```python
from build123d import *


with BuildPart() as part:
    # Sketch1 → Revolve1 (revolve)
    with BuildSketch(Plane.XY):
        Polygon((0, 0), (0, 3.5), (3.91, 3.5), (3.91, 1.4), (32.91, 1.4), (32.91, 1.9), (38.91, 1.9), (38.91, 0), align=None)
    revolve(axis=Axis((38.91, 0, 0), (-1, 0, 0)))


solid = part.part
```
Geometry check sheet. Reference: the model listing, model coordinates, mm. A direction names the side the tool comes from. Round coordinates to 2 decimals unless told otherwise and drop trailing zeros. Order: outer loops, then holes, each group sorted by start corner. A loop starts at its lowest first (then second) coordinate and runs counter-clockwise, first axis right, second up. Notation, with made-up numbers: M 19,-5.75 L 77,-5.75 A5 cw 77,2.25 Z; hole C 86.25,-9 d5. An arc over 180 degrees is marked long. Write item = value, one per line.
Q1. Section check D-D (z = 3). Enter the section's corners in (x, y).
Answer block:
outline = M 0,-1.8 L 3.91,-1.8 L 3.91,1.8 L 0,1.8 Z
Q2. Set-up check for faces 1 (the flat face through (3.91, 0, 2)), 2 (the cylindrical face through (35.95, -1.9, -0.08)): record each of +Z, -Z, +X, -X, +Y, -Y from which the full face is reachable in a straight line by a thin tool's end or side.
Answer block:
face_1 = none
face_2 = +X
Q3. Scan lines: line 1 (X direction, y = -1.5, z = -1); line 2 (X direction, y = 2, z = -2.25); line 3 (Z direction, x = 13, y = -1.25). Record each from-to range of solid material in increasing order.
Answer block:
line_1 = 0 to 3.91, 32.91 to 38.91
line_2 = 0 to 3.91
line_3 = -0.63 to 0.63
Q4. Depth check by flat-ended pin: pin 1 Ø3 at (x, y) = (12.5, -2.5) entering from -Z; pin 2 Ø2 at (x, z) = (5, 0.5) entering from -Y. Enter the tip coordinate at first touch or a pass-through.
Answer block:
pin_1 = -0.98
pin_2 = -1.4
Q5. Section check A-A (z = 0). Enter the section's corners in (x, y).
Answer block:
outline = M 0,-3.5 L 3.91,-3.5 L 3.91,-1.4 L 32.91,-1.4 L 32.91,-1.9 L 38.91,-1.9 L 38.91,1.9 L 32.91,1.9 L 32.91,1.4 L 3.91,1.4 L 3.91,3.5 L 0,3.5 Z
Q6. Release check for a two-part mould opening along X. For faces 3 (the cylindrical face through (18.61, -1.4, -0.06)), 4 (the cylindrical face through (1.982, 3.233, 1.341)), 5 (the flat face through (38.91, 0, 0)), 6 (the flat face through (0, 0, 0)) record: released by +X, released by -X, zero draft, split by the parting line, or undercut.
Answer block:
face_3 = undercut
face_4 = zero draft
face_5 = released by +X
face_6 = released by -X
Q7. Section check C-C (x = 5.5). Enter the section's corners in (y, z), plus the area to 3 significant figures.
Answer block:
outline = C 0,0 d2.8
area = 6.16 mm^2
